Build history of the part. All positions in model axes, mm. A direction names the side the tool comes from. Give positions to 0.01 mm unless a question says otherwise; leave off trailing zeros. Order: outer loops, then holes, each group sorted by start corner. A loop starts at its lowest first (then second) coordinate and runs counter-clockwise, first axis right, second up. Notation, with made-up numbers: (72.25, 31) - (97.25, 31) arc R24 cw to (97.25, 53) - close; hole circle Ø3 at (-27.75, -37). An arc over 180 degrees is marked (long way). Write each question's results on one line, items separated by ' | '. Start each with the question number.
1) Cut at B-B on z = -57. List the corners of the cut face in (x, y).
2) Drill centre lines: line 1 along X through (y, z) = (2.9, -57); line 2 along Z through (x, y) = (-0.5, 4.5); line 3 along X through (y, z) = (5.6, -34.5). Where is each one in solid material? Low to high. Write a range as from..to.
3) Tool access for faces 4 (the face through (-11.87, 2.96, -27.22)), 5 (the face through (-12.86, 2.96, -27.08)): list every direction of +Z, -Z, +X, -X, +Y, -Y with a clear straight run to the whole face (end or side of a thin tool).
4) Two-plate mould, pull along X, no slides. Class faces 1 (the face through (12.75, 2.96, -26.3)), 2 (the face through (-0.179, 2.958, 8.952)), 3 (the face through (11.76, 2.96, -26.44)): +X half, -X half, draft (parallel to the pull), parting line (faces both ways), or undercut.
5) Cut at A-A on x = 0. List the corners of the cut face in (y, z), plus the area to 3 significant figures.
6) Drop flat-ended pins along their axis: pin 1 Ø1 at (y, z) = (3.5, -11) entering from -X; pin 2 Ø2 at (x, y) = (11, 2) entering from -Z; pin 3 Ø1 at (y, z) = (2.5, -58.5) entering from -X. Give the stop position or say it passes through.
7) Cut at C-C on y = 2.75. List the corners of the cut face in (x, z), plus the area to 3 significant figures.
from build123d import *

# Parameters (mm, degrees)
BOSS_EXTRUDE1_DEPTH = 6


with BuildPart() as part:
    # Sketch1 → Boss-Extrude1 (new body)
    with BuildSketch(Plane(origin=(0, 0, 0), x_dir=(1, 0, 0), z_dir=(0, 1, 0))):
        with BuildLine():
            Line((-16.748260586, 54.637974737), (-8.866260216, -1.250418246))
            ThreePointArc((-8.866260216, -1.250418246), (0, -8.954), (8.866260216, -1.250418246))
            Line((8.866260216, -1.250418246), (16.748260586, 54.637974737))
            ThreePointArc((16.748260586, 54.637974737), (0, 73.914), (-16.748260586, 54.637974737))
        make_face()
        with BuildLine():
            Line((-15.758059534, 54.77762386), (-7.876059164, -1.110769123))
            ThreePointArc((-7.876059164, -1.110769123), (0, -7.954), (7.876059164, -1.110769123))
            Line((7.876059164, -1.110769123), (15.758059534, 54.77762386))
            ThreePointArc((15.758059534, 54.77762386), (0, 72.914), (-15.758059534, 54.77762386))
        make_face(mode=Mode.SUBTRACT)
    extrude(amount=BOSS_EXTRUDE1_DEPTH)


solid = part.part
Results:
1) outline: (-16.91, 0) - (-15.91, 0) - (-15.91, 6) - (-16.91, 6) - close; (15.91, 0) - (16.91, 0) - (16.91, 6) - (15.91, 6) - close
2) line 1: -16.91..-15.91, 15.91..16.91 | line 2: -73.91..-72.91, 7.94..8.94 | line 3: -13.91..-12.9, 12.9..13.91
3) face 4: +Y, -Y | face 5: +Z, -X, +Y, -Y
4) face 1: +X half | face 2: parting line | face 3: undercut
5) outline: (0, -73.91) - (6, -73.91) - (6, -72.91) - (0, -72.91) - close; (0, 7.95) - (6, 7.95) - (6, 8.95) - (0, 8.95) - close | area: 12.0 mm^2
6) pin 1: x = -10.66 | pin 2: z = -70.64 | pin 3: x = -16.88
7) outline: (-16.75, -54.64) arc R16.91 ccw (long way) to (16.75, -54.64) - (8.87, 1.25) arc R8.95 ccw to (-8.87, 1.25) - close; hole (-15.76, -54.78) arc R15.91 ccw (long way) to (15.76, -54.78) - (7.88, 1.11) arc R7.95 ccw to (-7.88, 1.11) - close | area: 193 mm^2
